For this review, take the finished solid that the model builds, in its own axes (mm). A direction names the side the tool comes from. Coordinates: 2 decimals unless noted, no trailing zeros. Loops run counter-clockwise (first coordinate to the right, second up) from the corner with the lowest first, then second, coordinate; pieces in that order, holes last.
1. Clearance check with flat-ended pins moving along their axes: P1, Ø2, axis at x = 6, z = -11, coming from the +Y side; P2, Ø5, axis at x = 0, y = 0, coming from the -Z side; P3, Ø5, axis at x = -2, y = -0.5, coming from the -Z side. State where each tip first meets the part, or that it passes through.
2. Mouldability with a two-part tool opening along Z and no side actions: class faces 1 (the face through (-4, -6, -23)), 2 (the face through (-3, 0, -18)), 3 (the face through (0, -38, -47)), 4 (the face through (-0.651, -37.815, -45.043)) as pulls with the +Z half, pulls with the -Z half, needs draft (parallel to the pull), parting line crosses it, or undercut.
3. Take a section at A-A, the plane x = 0. State the section outline as (y, z) points, then the cut area to 3 significant figures.
4. Take a section at B-B, the plane z = -7. State the section outline as (x, y) points, then the cut area to 3 significant figures.
5. Take a section at C-C, the plane y = -32.5. State the section outline as (x, z) points, then the cut area to 3 significant figures.
6. Machinability: for faces 5 (the face through (4.77, -1.5, -32.53)), 6 (the face through (6.466, -2.681, -11.661)), 7 (the face through (0.1, -60, -46.7)), which of the approach directions +Z, -Z, +X, -X, +Y, -Y give a long, thin tool a straight path to every point of the face, cutting with its end or side? Answer none if there is none.
7. To check wall thickness, follow probe 1 along Y at (x, z) = (0, -20.5); probe 2 along Z at (x, y) = (0, -36.5). State the ranges of each line that lie inside material, in increasing order.
```python
from build123d import *

# Parameters (mm, degrees)
SKETCH2_R           = 5
SKETCH2_R_2         = 3
BOSS_EXTRUDE1_START = -30
SKETCH3_R           = 7
SKETCH3_R_2         = 5
BOSS_EXTRUDE1_DEPTH = 30
SKETCH4_R           = 8
SKETCH4_R_2         = 7
BOSS_EXTRUDE2_DEPTH = 7


with BuildPart() as part:
    # Sweep1: sweep along a path in Sketch1
    with BuildLine(Plane(origin=(0, 0, 0), x_dir=(0, 0, -1), z_dir=(1, 0, 0))) as sweep1_path:
        Line((0, 0), (35, 0))
        ThreePointArc((35, 0), (45.606601718, -4.393398282), (50, -15))
        Line((50, -15), (50, -60))
    # Sketch2 → Sweep1 (sweep)
    with BuildSketch(Plane.XY):
        Circle(SKETCH2_R)
        Circle(SKETCH2_R_2, mode=Mode.SUBTRACT)
    sweep(path=sweep1_path.line)

    # Sketch3 → Boss-Extrude1 (add)
    with BuildSketch(Plane.XY.offset(BOSS_EXTRUDE1_START)):
        Circle(SKETCH3_R)
        with Locations(Location((0, 0, 0), (0, 0, 90))):
            Circle(SKETCH3_R_2, mode=Mode.SUBTRACT)
    extrude(amount=BOSS_EXTRUDE1_DEPTH)

    # Sketch4 → Boss-Extrude2 (add)
    with BuildSketch(Plane(origin=(0, 0, -30), x_dir=(-1, 0, 0), z_dir=(0, 0, -1))):
        Circle(SKETCH4_R)
        with Locations(Location((0, 0, 0), (0, 0, 180))):
            Circle(SKETCH4_R_2, mode=Mode.SUBTRACT)
    extrude(amount=-BOSS_EXTRUDE2_DEPTH)


solid = part.part
```
Results list:
1. P1: stops at y = 4.9
1. P2: stops at z = -50.61
1. P3: stops at z = -50.72
2. face 1: pulls with the +Z half
2. face 2: needs draft
2. face 3: undercut
2. face 4: parting line crosses it
3. outline: (-60, -55) - (-15, -55) arc R20 ccw to (5, -35) - (5, -30) - (8, -30) - (8, -23) - (7, -23) - (7, 0) - (3, 0) - (3, -35) arc R18 cw to (-15, -53) - (-60, -53) - close; (-60, -47) - (-15, -47) arc R12 ccw to (-3, -35) - (-3, 0) - (-7, 0) - (-7, -23) - (-8, -23) - (-8, -30) - (-5, -30) - (-5, -35) arc R10 cw to (-15, -45) - (-60, -45) - close
3. area: 548 mm2
4. outline: circle Ø14 at (0, 0); hole circle Ø6 at (0, 0)
4. area: 126 mm2
5. outline: circle Ø10 at (0, -50); hole circle Ø6 at (0, -50)
5. area: 50.3 mm2
6. face 5: none
6. face 6: +Z
6. face 7: +Z, -Z, +X, -X, -Y
7. probe 1: y = -7 to -3, 3 to 7
7. probe 2: z = -55 to -53, -47 to -45
